from build123d import *

# Parameters (mm, degrees)
SKETCH1_R           = 24.5
SKETCH1_R_2         = 15
BOSS_EXTRUDE1_DEPTH = 0.5
SKETCH2_R           = 2.5
CUT_EXTRUDE1_DEPTH  = 0.5


with BuildPart() as part:
    # Sketch1 → Boss-Extrude1 (new body)
    with BuildSketch(Plane.XY):
        Circle(SKETCH1_R)
        Circle(SKETCH1_R_2, mode=Mode.SUBTRACT)
    extrude(amount=BOSS_EXTRUDE1_DEPTH)

    # Sketch2 → Cut-Extrude1 (cut)
    with BuildSketch(Plane.XY.offset(0.5)):
        with Locations((0, 20)):
            Circle(SKETCH2_R)
        with Locations((17.320508076, -10)):
            Circle(SKETCH2_R)
        with Locations((-17.320508076, -10)):
            Circle(SKETCH2_R)
    extrude(amount=-CUT_EXTRUDE1_DEPTH, mode=Mode.SUBTRACT)


solid = part.part
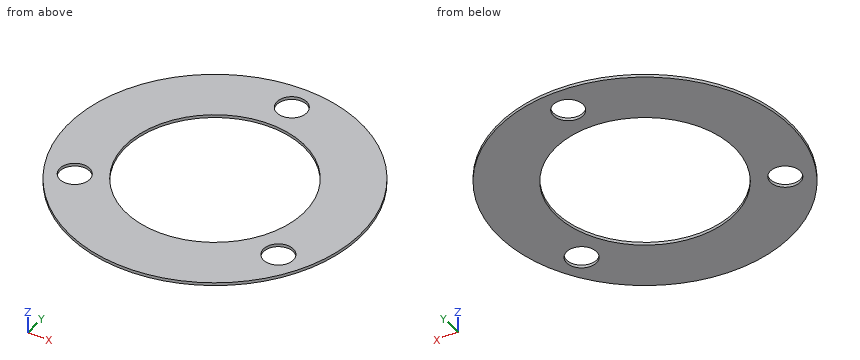
Model file for the job. Use its own axes, mm. Give positions to 0.01 mm unless a question says otherwise; leave off trailing zeros. Order: outer loops, then holes, each group sorted by start corner. A loop starts at its lowest first (then second) coordinate and runs counter-clockwise, first axis right, second up. Notation, with made-up numbers: M 13,39.5 L 24,39.5 A13 cw 24,45.5 Z; hole C 61,47.25 d11. An arc over 180 degrees is marked long. Put each result on its own line as item: value. Start each with the question number.
(1) Drill centre lines: L1, parallel to Y at x = 0, z = 0.35; L2, parallel to Y at x = -4, z = 0.05; L3, parallel to Y at x = -13, z = 0.4. Where is each one in solid material? Low to high. Write a range as [from, to].
(2) Band-saw the part on C-C on z = 0.4. Give the cut face in (x, y).
(3) Band-saw the part on B-B on y = 0. Give the cut face in (x, z).
(4) Band-saw the part on D-D on x = -8. Give the cut face in (y, z), then the cut area to 3 significant figures.
(5) Band-saw the part on A-A on x = 0. Give the cut face in (y, z), then the cut area to 3 significant figures.
Results below:
1. L1: y = [-24.5, -15], [15, 17.5], [22.5, 24.5]
1. L2: y = [-24.17, -14.46], [14.46, 24.17]
1. L3: y = [-20.77, -7.48], [7.48, 20.77]
2. outline: C 0,0 d49; hole C -17.32,-10 d5; hole C 0,0 d30; hole C 0,20 d5; hole C 17.32,-10 d5
3. outline: M -24.5,0 L -15,0 L -15,0.5 L -24.5,0.5 Z; M 15,0 L 24.5,0 L 24.5,0.5 L 15,0.5 Z
4. outline: M -23.16,0 L -12.69,0 L -12.69,0.5 L -23.16,0.5 Z; M 12.69,0 L 23.16,0 L 23.16,0.5 L 12.69,0.5 Z
4. area: 10.5 mm2
5. outline: M -24.5,0 L -15,0 L -15,0.5 L -24.5,0.5 Z; M 15,0 L 17.5,0 L 17.5,0.5 L 15,0.5 Z; M 22.5,0 L 24.5,0 L 24.5,0.5 L 22.5,0.5 Z
5. area: 7.00 mm2
